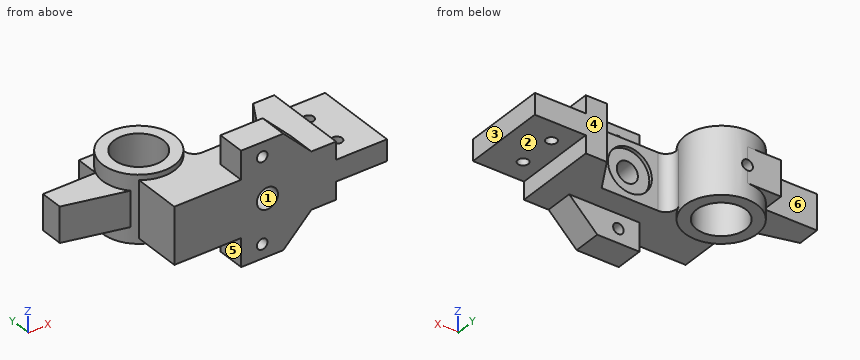
from build123d import *

# Parameters (mm, degrees)
BASE_BLOCK_SKETCH_R              = 20.5
BASE_BLOCK_SKETCH_R_2            = 14
BASE_BLOCK_DEPTH                 = 19
JOURNAL_HOUSING_PROFILE_SKETCH_R = 3
JOURNAL_HOUSING_DEPTH            = 16
HOUSING_FILLET_R6_R              = 6
MOUNTING_FLANGE_DEPTH            = 16
HOUSING_CUT_SKETCH_W             = 29
HOUSING_CUT_SKETCH_H             = 10
HOUSING_CUT_DEPTH                = 124.324774478
FLANGE_HOLES_SKETCH_R            = 3
FLANGE_HOLES_2X_6_DEPTH          = 16
COUNTERBORED_HOLE_12_D           = 12
COUNTERBORED_HOLE_12_DEPTH       = 99.788526395
COUNTERBORED_HOLE_12_CBORE_D     = 25
COUNTERBORED_HOLE_12_CBORE_DEPTH = 2
SIDE_LUG_DEPTH                   = 10
LUG_HOLE_6_REACH                 = 132.634
LUG_HOLE_6_END_RADIUS            = 14
LUG_HOLE_SKETCH_R                = 3


with BuildPart() as part:
    # Base Block Sketch → Base Block (new, symmetric)
    with BuildSketch(Plane.XY):
        Circle(BASE_BLOCK_SKETCH_R)
        Circle(BASE_BLOCK_SKETCH_R_2, mode=Mode.SUBTRACT)
    extrude(amount=BASE_BLOCK_DEPTH, both=True)

    # Journal Housing Profile Sketch → Journal Housing (add, symmetric)
    with BuildSketch(Plane.XY):
        Polygon((-12, -44), (-12, -15), (57.030344885, -15), (68, 4), (109, 4), (109, -44), align=None)
        with Locations((90, -31)):
            Circle(JOURNAL_HOUSING_PROFILE_SKETCH_R, mode=Mode.SUBTRACT)
        with Locations((90, -9)):
            Circle(JOURNAL_HOUSING_PROFILE_SKETCH_R, mode=Mode.SUBTRACT)
    extrude(amount=JOURNAL_HOUSING_DEPTH, both=True)

    # Housing Fillet R6
    housing_fillet_r6_edges = [part.edges().sort_by_distance(p)[0] for p in [
        (13.973188612, -15, 0),
    ]]
    fillet(housing_fillet_r6_edges, radius=HOUSING_FILLET_R6_R)

    # Mounting Flange Sketch → Mounting Flange (add)
    with BuildSketch(Plane.XZ.offset(44)):
        Polygon((26, 16), (26, 32), (50, 32), (66, 16), align=None)
        Polygon((50, -32), (66, -16), (26, -16), (26, -32), align=None)
    extrude(amount=-MOUNTING_FLANGE_DEPTH)

    # Housing Cut Sketch → Housing Cut (cut, through all)
    with BuildSketch(Plane(origin=(0, 4, 0), x_dir=(1, 0, 0), z_dir=(0, 1, 0))):
        with Locations((94.5, -11)):
            Rectangle(HOUSING_CUT_SKETCH_W, HOUSING_CUT_SKETCH_H)
        with Locations((94.5, 11)):
            Rectangle(HOUSING_CUT_SKETCH_W, HOUSING_CUT_SKETCH_H)
    extrude(amount=-HOUSING_CUT_DEPTH, mode=Mode.SUBTRACT)

    # Flange Holes Sketch → Flange Holes 2xØ6 (cut)
    with BuildSketch(Plane(origin=(0, -28, 0), x_dir=(1, 0, 0), z_dir=(0, 1, 0))):
        with Locations(Location((38, -24, 0), (0, 0, 180))):
            Circle(FLANGE_HOLES_SKETCH_R)
        with Locations((38, 24)):
            Circle(FLANGE_HOLES_SKETCH_R)
    extrude(amount=-FLANGE_HOLES_2X_6_DEPTH, mode=Mode.SUBTRACT)

    # Counterbored Hole Ø12
    with Locations(Plane(origin=(40.977616023, -15, 0), x_dir=(0, 0, 1), z_dir=(0, 1, 0))):
        with Locations((0, 0)):
            CounterBoreHole(COUNTERBORED_HOLE_12_D / 2, COUNTERBORED_HOLE_12_CBORE_D / 2, COUNTERBORED_HOLE_12_CBORE_DEPTH, depth=COUNTERBORED_HOLE_12_DEPTH)

    # Side Lug Sketch → Side Lug (add, symmetric)
    with BuildSketch(Plane.XY):
        with BuildLine():
            Line((0, 20.5), (-19, 20.5))
            Line((-19, 20.5), (-19, 7.5))
            Line((-19, 7.5), (-49, 7.5))
            Line((-49, 7.5), (-49, -5.5))
            Line((-49, -5.5), (-13.090107344, -14.453341818))
            ThreePointArc((-13.090107344, -14.453341818), (-18.194644342, 7.014621677), (0, 19.5))
            Line((0, 19.5), (0, 20.5))
        make_face()
    extrude(amount=SIDE_LUG_DEPTH, both=True)

    # Lug Hole Ø6: up to this cylinder (the profile starts outside it)
    lug_hole_6_end = Plane(origin=(0, 0, 0), z_dir=(0, 0, -1)) * Cylinder(LUG_HOLE_6_END_RADIUS, 294.268, mode=Mode.PRIVATE)
    # Lug Hole Sketch → Lug Hole Ø6 (cut, up to the surface)
    with BuildSketch(Plane(origin=(0, 20.5, 0), x_dir=(1, 0, 0), z_dir=(0, 1, 0)), mode=Mode.PRIVATE) as lug_hole_6_sk1:
        with Locations(Location((0, 0, 0), (0, 0, 270))):
            Circle(LUG_HOLE_SKETCH_R)
    lug_hole_6_tool1 = extrude(lug_hole_6_sk1.sketch, amount=-LUG_HOLE_6_REACH, mode=Mode.PRIVATE) - lug_hole_6_end
    add(lug_hole_6_tool1.solids().sort_by_distance((0, 20.5, 0))[0], mode=Mode.SUBTRACT)


solid = part.part
Design review of the part built by this model. Coordinates are the model's own, in mm. Face numbers are marked on the shaded views. A direction names the side the tool comes from. Give positions to 0.01 mm unless a question says otherwise; leave off trailing zeros. Write each loop counter-clockwise with the first axis right and the second up, starting at its lowest first coordinate (ties: lowest second). Pieces come first, ordered by that corner, then holes. Notation, with made-up numbers: M 61.25,-14.75 L 72.25,-14.75 A23 cw 72.25,2.25 Z; hole C 65.25,4 d8. An arc over 180 degrees is marked long. Return JSON: item names as keys, results as strings. Group by question number.
Item 1: Take a section at B-B (y = 5.5). Give the boundary of the cut face in (x, z).
Item 2: Take a section at C-C (x = 38.5). Give the boundary of the cut face in (y, z), plus the area to 3 significant figures.
Item 3: Take a section at A-A (z = 24). Give the boundary of the cut face in (x, y), plus the area to 3 significant figures.
Item 4: Tool access review of the marked faces 4, 5 and 6: name each direction out of +Z, -Z, +X, -X, +Y, -Y from which nothing blocks a thin tool from reaching the whole face with its end or side.
Item 5: Take a section at D-D (z = 0). Give the boundary of the cut face in (x, y).
Item 6: Wall thickness on line 1 along Y through (x, z) = (90, 0); line 2 along X through (y, z) = (-1, -5); line 3 along Y through (x, z) = (35.5, -28): over which ranges is each line inside the solid? List them lowest first.
Item 7: The part is to be moulded in two halves that separate along Z. For the marked faces 1, 2 and 3, say which applies: pulls with the +Z half, pulls with the -Z half, needs draft (parallel to the pull), parting line crosses it, or undercut.
Item 8: Clearance check with flat-ended pins moving along their axes: pin 1 Ø6.5 at (x, y) = (-39.5, -5) entering from +Z; pin 2 Ø13 at (x, z) = (49, 25) entering from +Y; pin 3 Ø4 at (x, y) = (14.5, -11) entering from +Z; pin 4 Ø5 at (x, z) = (38, -24) entering from -Y. State where each tip first meets the part, or that it passes through.
Return value:
{
 "1": {"outline": "M -49,-10 L -19.75,-10 L -19.75,-19 L -12.87,-19 L -12.87,19 L -19.75,19 L -19.75,10 L -49,10 Z; M 12.87,-19 L 19.75,-19 L 19.75,19 L 12.87,19 Z"},
 "2": {"outline": "M -44,-32 L -28,-32 L -28,-26.96 L -44,-26.96 Z; M -44,-21.04 L -28,-21.04 L -28,-16 L -15,-16 L -15,-12.25 L -17,-12.25 L -17,-5.46 L -44,-5.46 Z; M -44,5.46 L -17,5.46 L -17,12.25 L -15,12.25 L -15,16 L -28,16 L -28,21.04 L -44,21.04 Z; M -44,26.96 L -28,26.96 L -28,32 L -44,32 Z", "area": "907 mm2"},
 "3": {"outline": "M 26,-44 L 35,-44 L 35,-28 L 26,-28 Z; M 41,-44 L 58,-44 L 58,-28 L 41,-28 Z", "area": "416 mm2"},
 "4": {"face 4": "+Z, -Z, +X, +Y", "face 5": "-Z, -X, +Y, -Y", "face 6": "+Z, -Z, -X, +Y"},
 "5": {"outline": "M -49,-5.5 L -15,-13.98 A20.5 ccw -12,-16.62 L -12,-44 L 34.98,-44 L 34.98,-17 L 28.48,-17 L 28.48,-15 L 24.92,-15 A6 cw 19.28,-6.96 A20.5 ccw 3,20.28 L 3,13.67 A14 cw long -3,13.67 L -3,20.5 L -19,20.5 L -19,7.7 A20.5 ccw -19.08,7.5 L -49,7.5 Z; M 46.98,-44 L 109,-44 L 109,4 L 68,4 L 57.03,-15 L 53.48,-15 L 53.48,-17 L 46.98,-17 Z; hole C 90,-31 d6; hole C 90,-9 d6"},
 "6": {"line 1": "y = -44 to -34, -28 to -12, -6 to 4", "line 2": "x = -49 to -13.96, 13.96 to 20.48, 65.11 to 109", "line 3": "y = -44 to -28"},
 "7": {"face 1": "undercut", "face 2": "pulls with the -Z half", "face 3": "needs draft"},
 "8": {"pin 1": "stops at z = 10", "pin 2": "stops at y = -28", "pin 3": "stops at z = 19", "pin 4": "passes through"}
}
